Build history of the part. All positions in model axes, mm. A direction names the side the tool comes from. Give positions to 0.01 mm unless a question says otherwise; leave off trailing zeros. Order: outer loops, then holes, each group sorted by start corner. A loop starts at its lowest first (then second) coordinate and runs counter-clockwise, first axis right, second up. Notation, with made-up numbers: (-26, 26) -> (-13, 26) arc R27 ccw to (-13, 55) -> close; hole circle Ø4 at (-5, 23). An arc over 180 degrees is marked (long way). One line per question, with ' | ' between items. Start each with the question number.
(1) Drill centre lines: L1, parallel to X at y = 0, z = 3.25; L2, parallel to X at y = 1.25, z = 11.5; L3, parallel to Y at x = 137, z = -5.25. Where is each one in solid material? Low to high. Write a range as from..to.
(2) Cut at C-C (x = 44). Give the cut face in (y, z), then the cut area to 3 significant figures.
(3) Pin check, flat tips, straight feed: pin 1 Ø6.5 at (x, y) = (137, 0) entering from -Z; pin 2 Ø2 at (x, y) = (104.5, 9.5) entering from +Z; pin 3 Ø3 at (x, y) = (94.5, -3.5) entering from -Z. Stop position of each tip, or through.
(4) Cut at D-D (x = 137). Give the cut face in (y, z), then the cut area to 3 significant figures.
(5) Pull direction X, two halves, no side cores. Call faces 3 (the face through (0, 0, 0)), 4 (the face through (3.48, -12.65, -8.06)), 5 (the face through (144.81, -2.34, -7.44)), 6 (the face through (139.385, 0.751, -0.14)): +X half, -X half, draft (parallel to the pull), parting line (faces both ways), or undercut.
(6) Cut at A-A (y = 0). Give the cut face in (x, z).
(7) Which spindle directions (+Z, -Z, +X, -X, +Y, -Y) get a long thin tool onto all of the face, cutting with end or side? Do faces 1 (the face through (145, 0, 0)), 2 (the face through (5, -10, -5)). Say none if no direction does.
(8) Cut at B-B (z = 0). Give the cut face in (x, y), then the cut area to 3 significant figures.
from build123d import *

# Parameters (mm, degrees)
CUT_EXTRUDE_1_DEPTH      = 147.543508898
CUT_EXTRUDE_1_DEPTH_BACK = 147.543508898
SKETCH_2_R               = 2.5
FILLET_1_R               = 1
CHAMFER_1_SIZE           = 4
CHAMFER_1_SIZE2          = 2.309401077


with BuildPart() as part:
    # 草图1 → Revolve 546 (revolve)
    with BuildSketch(Plane.XY, mode=Mode.PRIVATE) as revolve_546_sk:
        Polygon((0, 0), (145, 0), (145, 10), (5, 10), (5, 15), (2, 15), (0, 13), align=None)
    revolve(revolve_546_sk.sketch.rotate(Axis((0, 0, 0), (-1, 0, 0)), 90), axis=Axis((0, 0, 0), (-1, 0, 0)))

    # 草图2 → 切除-拉伸1 (cut, two sides: drawn at the far end of the back side and taken through both)
    with BuildSketch(Plane.XY.offset(-CUT_EXTRUDE_1_DEPTH_BACK)):
        with Locations((137, 0)):
            Circle(SKETCH_2_R)
    extrude(amount=CUT_EXTRUDE_1_DEPTH + CUT_EXTRUDE_1_DEPTH_BACK, mode=Mode.SUBTRACT)

    # 圆角1
    fillet_1_edges = [part.edges().sort_by_distance(p)[0] for p in [
        (5, 0, 10),
    ]]
    fillet(fillet_1_edges, radius=FILLET_1_R)

    # 倒角1
    chamfer_1_edges = [part.edges().sort_by_distance(p)[0] for p in [
        (145, 0, 10),
    ]]
    chamfer_1_side = [part.faces().sort_by_distance(p)[0] for p in [
        (75.5, 0, 10),
    ]]
    chamfer(chamfer_1_edges, length=CHAMFER_1_SIZE, length2=CHAMFER_1_SIZE2, reference=chamfer_1_side[0])


solid = part.part
Result set:
1) L1: x = 0..134.5, 139.5..145 | L2: x = 0..5 | L3: y = -8.51..-2.5, 2.5..8.51
2) outline: circle Ø20 at (0, 0) | area: 314 mm2
3) pin 1: stops at z = -10 | pin 2: stops at z = 5.27 | pin 3: stops at z = -9.8
4) outline: (-2.5, -9.68) -> (-2.5, 9.68) arc R10 ccw to start; (2.5, -9.68) arc R10 ccw to (2.5, 9.68) -> close | area: 215 mm2
5) face 3: -X half | face 4: draft | face 5: +X half | face 6: undercut
6) outline: (0, -13) -> (2, -15) -> (5, -15) -> (5, -11) arc R1 cw to (6, -10) -> (134.5, -10) -> (134.5, 10) -> (6, 10) arc R1 cw to (5, 11) -> (5, 15) -> (2, 15) -> (0, 13) -> close; (139.5, -10) -> (141, -10) -> (145, -7.69) -> (145, 7.69) -> (141, 10) -> (139.5, 10) -> close
7) face 1: +Z, -Z, +X, +Y, -Y | face 2: +X
8) outline: (0, -13) -> (2, -15) -> (5, -15) -> (5, -11) arc R1 cw to (6, -10) -> (141, -10) -> (145, -7.69) -> (145, 7.69) -> (141, 10) -> (6, 10) arc R1 cw to (5, 11) -> (5, 15) -> (2, 15) -> (0, 13) -> close; hole circle Ø5 at (137, 0) | area: 2,920 mm2
